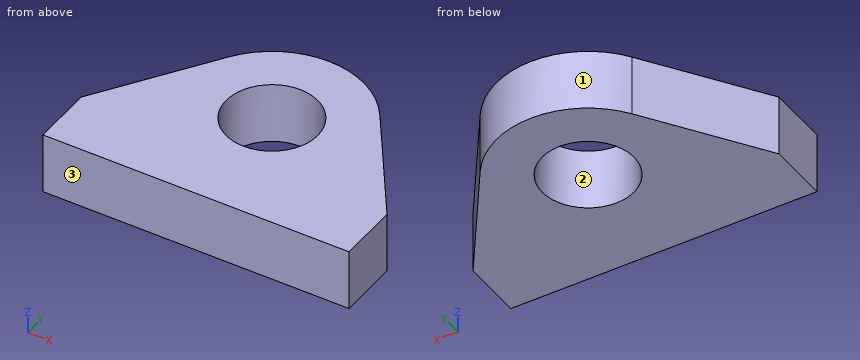
from build123d import *

# Parameters (mm, degrees)
SKETCH_1_R      = 7.5
EXTRUDE_1_DEPTH = 10


with BuildPart() as part:
    # 草图1 → 凸台-拉伸1 (new body)
    with BuildSketch(Plane.XY):
        with BuildLine():
            Line((25, -20), (-25, -20))
            Line((-25, -20), (-25, -10))
            Line((-25, -10), (-12.384968229, 8.462420573))
            ThreePointArc((-12.384968229, 8.462420573), (0, 15), (12.384968229, 8.462420573))
            Line((12.384968229, 8.462420573), (25, -10))
            Line((25, -10), (25, -20))
        make_face()
        Circle(SKETCH_1_R, mode=Mode.SUBTRACT)
    extrude(amount=EXTRUDE_1_DEPTH)


solid = part.part
The listing builds one solid part. Answer for the finished solid, in the listing's coordinates (mm). Face numbers are marked on the shaded views. Coordinates: 2 decimals unless noted, no trailing zeros. Loops run counter-clockwise (first coordinate to the right, second up) from the corner with the lowest first, then second, coordinate; pieces in that order, holes last. Notation, with made-up numbers: (89, -39) -> (128, -39) arc R11 cw to (128, -35) -> close; hole circle Ø2 at (-24.5, -20.75). An arc over 180 degrees is marked (long way). Answer in a Markdown table with one row per item. Add a question column.
1. The part is cut by section C-C, the plane y = -1.5. Write down the section's boundary in (x, z).
2. The part is cut by section D-D, the plane y = 10.5. Write down the section's boundary in (x, z), then the cut area to 3 significant figures.
3. Consider line 1 (Y direction, x = 0, z = 4.25); line 2 (Y direction, x = -2.5, z = 7.5); line 3 (X direction, y = -4, z = 9). Determine where each line is inside the solid, lowest interval first. Write a range as [from, to].
4. Flat-ended cylindrical pins translate along their axes: P1, Ø3, axis at y = 4, z = 5.5, coming from the +X side; P2, Ø2, axis at x = 12, y = 2.5, coming from the -Z side; P3, Ø1.5, axis at y = -8.5, z = 1, coming from the -X side. Find the tip coordinate at first contact, or state that the pin passes through.
5. The part is cut by section B-B, the plane x = 0. Write down the section's boundary in (y, z).
6. The part is cut by section A-A, the plane z = 1.25. Write down the section's boundary in (x, y).
7. Determine the mould class of the marked faces 1, 2 and 3 for opening direction X: +X half, -X half, draft (parallel to the pull), parting line (faces both ways), or undercut.
Answer below:
| question | item | result |
|---|---|---|
| 1 | outline | (-19.19, 0) -> (-7.35, 0) -> (-7.35, 10) -> (-19.19, 10) -> close; (7.35, 0) -> (19.19, 0) -> (19.19, 10) -> (7.35, 10) -> close |
| 2 | outline | (-10.71, 0) -> (10.71, 0) -> (10.71, 10) -> (-10.71, 10) -> close |
| 2 | area | 214 mm2 |
| 3 | line 1 | [-20, -7.5], [7.5, 15] |
| 3 | line 2 | [-20, -7.07], [7.07, 14.79] |
| 3 | line 3 | [-20.9, -6.34], [6.34, 20.9] |
| 4 | P1 | x = 16.46 |
| 4 | P2 | z = 0 |
| 4 | P3 | x = -24.49 |
| 5 | outline | (-20, 0) -> (-7.5, 0) -> (-7.5, 10) -> (-20, 10) -> close; (7.5, 0) -> (15, 0) -> (15, 10) -> (7.5, 10) -> close |
| 6 | outline | (-25, -20) -> (25, -20) -> (25, -10) -> (12.38, 8.46) arc R15 ccw to (-12.38, 8.46) -> (-25, -10) -> close; hole circle Ø15 at (0, 0) |
| 7 | face 1 | parting line |
| 7 | face 2 | undercut |
| 7 | face 3 | draft |
